Verification items for this drawing (mm, ordinates from the low corner). Give positions to 0.01 mm unless a question says otherwise; leave off trailing zeros. Write each loop counter-clockwise with the first axis right and the second up, starting at its lowest first coordinate (ties: lowest second). Pieces come first, ordered by that corner, then holes. Notation, with made-up numbers: (83.5, -21) -> (134.5, -21) arc R16 cw to (134.5, -1) -> close; hole circle Ø1 at (86.5, 79). An arc over 180 degrees is marked (long way). Answer as a JSON object with one key per item and string values.
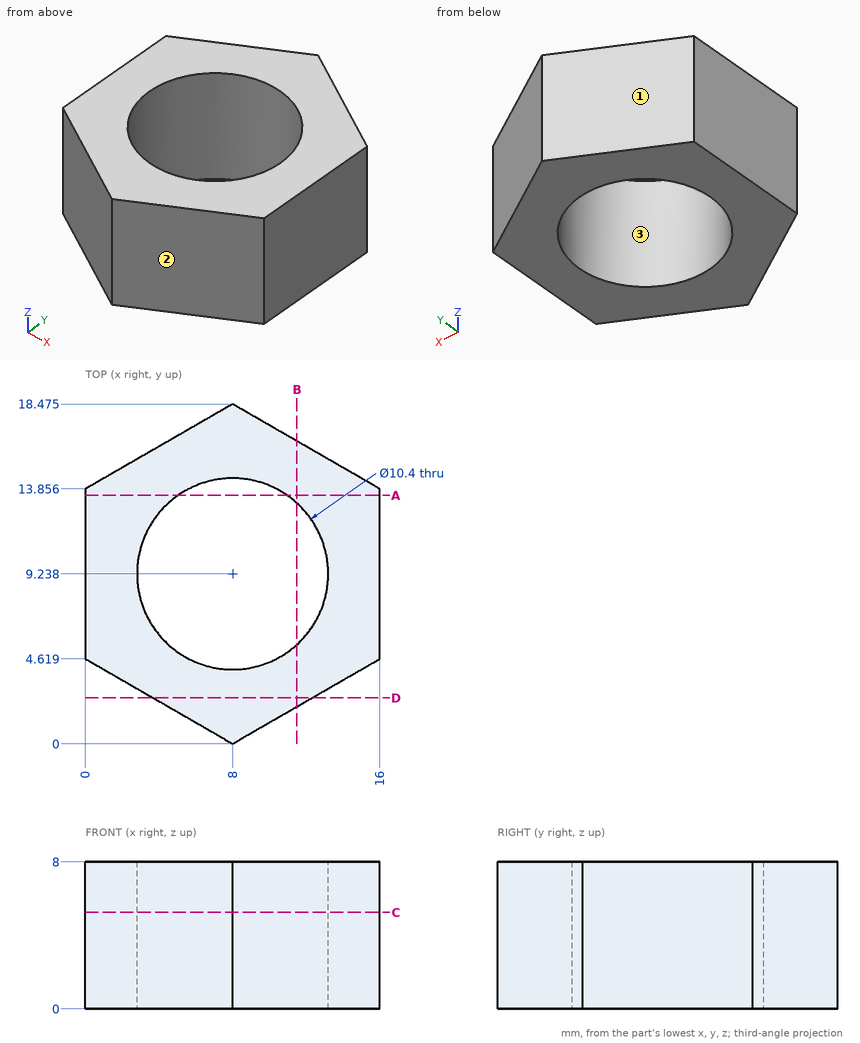
1. Scan lines: L1, parallel to X at y = 12.75, z = 0.5 (1 decimal); L2, parallel to Y at x = 8.25, z = 5.75 (1 decimal); L3, parallel to Y at x = 10, z = 7.5 (1 decimal). Record each from-to range of solid material in increasing order. Write a range as [from, to].
Determined:
{"L1": "[0, 4.2], [11.8, 16]", "L2": "[0.1, 4], [14.4, 18.3]", "L3": "[1.2, 4.4], [14, 17.3]"}
2. Sectioned sample at B-B, the plane x = 11.5. Enter the section's corners in (y, z) (1 decimal).
Determined:
{"outline": "(2, 0) -> (5.4, 0) -> (5.4, 8) -> (2, 8) -> close; (13.1, 0) -> (16.5, 0) -> (16.5, 8) -> (13.1, 8) -> close"}
3. Go/stop test with flat-tipped pins: P1, Ø4, axis at x = 11, z = 4, coming from the +Y side; P2, Ø1, axis at y = 4, z = 1.5, coming from the +X side (1 decimal); P3, Ø4, axis at y = 2.5, z = 1, coming from the -X side (1 decimal). Record where each tip stops, or that it passes through.
Determined:
{"P1": "y = 17.9", "P2": "x = 15.8", "P3": "x = 0.2"}
4. Sectioned sample at D-D, the plane y = 2.5. Enter the section's corners in (x, z).
Determined:
{"outline": "(3.67, 0) -> (12.33, 0) -> (12.33, 8) -> (3.67, 8) -> close"}
5. Mould release check, pull along Y, two halves, no side actions. Record for the marked faces 1, 2 and 3: released by +Y, released by -Y, zero draft, split by the parting line, or undercut.
Determined:
{"face 1": "released by +Y", "face 2": "released by -Y", "face 3": "undercut"}
6. Sectioned sample at A-A, the plane y = 13.5. Enter the section's corners in (x, z).
Determined:
{"outline": "(0, 0) -> (5.02, 0) -> (5.02, 8) -> (0, 8) -> close; (10.98, 0) -> (16, 0) -> (16, 8) -> (10.98, 8) -> close"}
7. Sectioned sample at C-C, the plane z = 5.25. Enter the section's corners in (x, y) (1 decimal).
Determined:
{"outline": "(0, 4.6) -> (8, 0) -> (16, 4.6) -> (16, 13.9) -> (8, 18.5) -> (0, 13.9) -> close; hole circle Ø10.4 at (8, 9.2)"}
